from build123d import *

# Parameters (mm, degrees)
SIDE_WINDOW_CUT_DEPTH      = 114.549548656
SIDE_WINDOW_CUT_DEPTH_BACK = 114.549548656
EDGE_FILLET_R2_R           = 2
BORE_16_REACH              = 115.55
BORE_16_END_RADIUS         = 9
BORE_SKETCH_16_R           = 8


with BuildPart() as part:
    # Holder Profile Sketch → Holder Body Revolve (revolve)
    with BuildSketch(Plane.XY, mode=Mode.PRIVATE) as holder_body_revolve_sk:
        Polygon((0, 0), (0, 22.5), (11, 22.5), (11, 16.5), (84, 16.5), (109, 12.5), (109, 0), align=None)
    revolve(holder_body_revolve_sk.sketch.rotate(Axis((-42.829787234, 0, 0), (1, 0, 0)), 90), axis=Axis((-42.829787234, 0, 0), (1, 0, 0)))

    # Side Window Sketch → Side Window Cut (cut, two sides: drawn at the far end of the back side and taken through both)
    with BuildSketch(Plane.XY.offset(-SIDE_WINDOW_CUT_DEPTH_BACK)):
        with BuildLine():
            Line((37, 9), (67, 9))
            ThreePointArc((67, 9), (76, 0), (67, -9))
            Line((67, -9), (37, -9))
            ThreePointArc((37, -9), (28, 0), (37, 9))
        make_face()
    extrude(amount=SIDE_WINDOW_CUT_DEPTH + SIDE_WINDOW_CUT_DEPTH_BACK, mode=Mode.SUBTRACT)

    # Edge Fillet R2
    edge_fillet_r2_edges = [part.edges().sort_by_distance(p)[0] for p in [
        (109, 0, -12.5),
    ]]
    fillet(edge_fillet_r2_edges, radius=EDGE_FILLET_R2_R)

    # Bore Ø16: up to this cylinder (the profile starts outside it)
    bore_16_end = Plane(origin=(67, 0, 0), z_dir=(0, 0, 1)) * Cylinder(BORE_16_END_RADIUS, 250.1, mode=Mode.PRIVATE)
    # Bore Sketch Ø16 → Bore Ø16 (cut, up to the surface)
    with BuildSketch(Plane(origin=(109, 0, 0), x_dir=(0, 0, -1), z_dir=(1, 0, 0)), mode=Mode.PRIVATE) as bore_16_sk1:
        Circle(BORE_SKETCH_16_R)
    bore_16_tool1 = extrude(bore_16_sk1.sketch, amount=-BORE_16_REACH, mode=Mode.PRIVATE) - bore_16_end
    add(bore_16_tool1.solids().sort_by_distance((109, 0, 0))[0], mode=Mode.SUBTRACT)


solid = part.part
Geometry check sheet. Reference: the model listing, model coordinates, mm. A direction names the side the tool comes from. Round coordinates to 2 decimals unless told otherwise and drop trailing zeros. Order: outer loops, then holes, each group sorted by start corner. A loop starts at its lowest first (then second) coordinate and runs counter-clockwise, first axis right, second up. Notation, with made-up numbers: M 53,89.5 L 80,89.5 A10 ccw 80,104.5 Z; hole C 0.5,-8 d1. An arc over 180 degrees is marked long. Write each question's results on one line, items separated by ' | '. Start each with the question number.
1. Cross-section at A-A on y = 0. Record the boundary of the cut face in (x, z), plus the area to 3 significant figures.
2. Cross-section at B-B on x = 74.5. Record the boundary of the cut face in (y, z).
3. Go/stop test with flat-tipped pins: P1, Ø2, axis at x = 25.5, y = 12, coming from the +Z side; P2, Ø8, axis at y = 16, z = 14, coming from the +X side; P3, Ø9.5, axis at y = 0, z = 0, coming from the +X side. Record where each tip stops, or that it passes through.
4. Material ranges on L1, parallel to Y at x = 96, z = 0; L2, parallel to Z at x = 88.5, y = -3; L3, parallel to Y at x = 54.5, z = 2, recorded low to high. Write a range as from..to.
5. Set-up check for faces 1 (the face through (0, 0, 0)), 2 (the face through (11, -12, -12)), 3 (the face through (52, -9, 0)): record each of +Z, -Z, +X, -X, +Y, -Y from which the full face is reachable in a straight line by a thin tool's end or side.
6. Draft check along Y on faces 4 (the face through (98.41, -4.26, 13.54)), 5 (the face through (28, 0, 0)), 6 (the face through (90.33, -3.06, -7.39)), 7 (the face through (109, 3.9, -7.2)). Enter one of: pulls with the +Y half, pulls with the -Y half, needs draft (parallel to the pull), parting line crosses it, or undercut.
7. Cross-section at C-C on x = 58.5. Record the boundary of the cut face in (y, z).
Resolved:
1) outline: M 0,-22.5 L 11,-22.5 L 11,-16.5 L 28,-16.5 L 28,16.5 L 11,16.5 L 11,22.5 L 0,22.5 Z; M 76,-16.5 L 84,-16.5 L 107.32,-12.77 A2 ccw 109,-10.79 L 109,-8 L 76,-8 Z; M 76,8 L 109,8 L 109,10.79 A2 ccw 107.32,12.77 L 84,16.5 L 76,16.5 Z | area: 1,520 mm2
2) outline: M -4.97,-15.73 L -4.97,-6.26 A8 cw -4.97,6.26 L -4.97,15.73 A16.5 ccw Z; M 4.97,-15.73 A16.5 ccw 4.97,15.73 L 4.97,6.26 A8 cw 4.97,-6.26 Z
3) P1: z = 12.3 | P2: x = 11 | P3: x = 29.36
4) L1: -14.58..-8, 8..14.58 | L2: -15.49..-7.42, 7.42..15.49 | L3: -16.38..-9, 9..16.38
5) face 1: +Z, -Z, -X, +Y, -Y | face 2: +X | face 3: +Z, -Z
6) face 4: parting line crosses it | face 5: undercut | face 6: undercut | face 7: needs draft
7) outline: M -9,-13.83 L -9,13.83 A16.5 ccw Z; M 9,-13.83 A16.5 ccw 9,13.83 Z
